The model under review builds one solid part; all positions refer to its coordinate system, in mm. Coordinates: 2 decimals unless noted, no trailing zeros. Order: outer loops, then holes, each group sorted by start corner. A loop starts at its lowest first (then second) coordinate and runs counter-clockwise, first axis right, second up. Notation, with made-up numbers: M -10.5,51.25 L 38.5,51.25 A26 cw 38.5,66.25 Z; hole C 78.5,47 d6. An arc over 180 degrees is marked long. Answer in a Markdown table with one row per item.
from build123d import *

# Parameters (mm, degrees)
BOSS_EXTRUDE1_DEPTH   = 7
SKETCH4_W             = 63
SKETCH4_H             = 38
CUT_EXTRUDE1_DEPTH    = 323.811382974
FILLET1_R             = 2
CUT_EXTRUDE2_DEPTH    = 323.811382974
FILLET2_R             = 2
M5_TAPPED_HOLE1_D     = 4.2
M5_TAPPED_HOLE1_DEPTH = 14
M5_TAPPED_HOLE1_TIP   = 1.2618073
M4_TAPPED_HOLE1_D     = 3.3
M4_TAPPED_HOLE1_DEPTH = 11.5
M4_TAPPED_HOLE1_TIP   = 0.991420021
FILLET3_R             = 3


with BuildPart() as part:
    # Sketch3 → Boss-Extrude1 (new, symmetric)
    with BuildSketch(Plane(origin=(50, 414.547428979, -101), x_dir=(0, 0, -1), z_dir=(-1, 0, 0))):
        Polygon((-101, 210.80448069), (-101, 290.80448069), (-262, 290.80448069), (-351, 227.80448069), (-351, 210.80448069), align=None)
    extrude(amount=BOSS_EXTRUDE1_DEPTH, both=True)

    # Sketch4 → Cut-Extrude1 (cut, through all)
    with BuildSketch(Plane(origin=(57, 0, 0), x_dir=(0, 0, -1), z_dir=(1, 0, 0))):
        with Locations((-46.5, 163.74294829)):
            Rectangle(SKETCH4_W, SKETCH4_H)
    extrude(amount=-CUT_EXTRUDE1_DEPTH, mode=Mode.SUBTRACT)

    # Fillet1
    fillet1_edges = [part.edges().sort_by_distance(p)[0] for p in [
        (50, 182.74294829, 15),
        (50, 144.74294829, 15),
        (50, 144.74294829, 78),
        (50, 182.74294829, 78),
    ]]
    fillet(fillet1_edges, radius=FILLET1_R)

    # Sketch5 → Cut-Extrude2 (cut, through all)
    with BuildSketch(Plane(origin=(57, 0, 0), x_dir=(0, 0, -1), z_dir=(1, 0, 0))):
        Polygon((-98, 144.74294829), (-157.507936508, 144.74294829), (-190, 167.74294829), (-190, 182.74294829), (-98, 182.74294829), align=None)
    extrude(amount=-CUT_EXTRUDE2_DEPTH, mode=Mode.SUBTRACT)

    # Fillet2
    fillet2_edges = [part.edges().sort_by_distance(p)[0] for p in [
        (50, 182.74294829, 98),
        (50, 144.74294829, 98),
        (50, 144.74294829, 157.507936508),
        (50, 167.74294829, 190),
        (50, 182.74294829, 190),
    ]]
    fillet(fillet2_edges, radius=FILLET2_R)

    # M5 Tapped Hole1
    with Locations(Plane(origin=(0, 0, 0), x_dir=(-1, 0, 0), z_dir=(0, 0, -1))):
        with Locations((-50.5, 188.74294829), (-50, 138.745448352)):
            Hole(M5_TAPPED_HOLE1_D / 2, depth=M5_TAPPED_HOLE1_DEPTH)
            with Locations((0, 0, -(M5_TAPPED_HOLE1_DEPTH + M5_TAPPED_HOLE1_TIP / 2))):  # 118° drill point
                Cone(0, M5_TAPPED_HOLE1_D / 2, M5_TAPPED_HOLE1_TIP, mode=Mode.SUBTRACT)

    # M4 Tapped Hole1
    with Locations(Plane(origin=(0, 203.74294829, 0), x_dir=(1, 0, 0), z_dir=(0, 1, 0))):
        with Locations((50, -114), (50, -174), (50, -234)):
            Hole(M4_TAPPED_HOLE1_D / 2, depth=M4_TAPPED_HOLE1_DEPTH)
            with Locations((0, 0, -(M4_TAPPED_HOLE1_DEPTH + M4_TAPPED_HOLE1_TIP / 2))):  # 118° drill point
                Cone(0, M4_TAPPED_HOLE1_D / 2, M4_TAPPED_HOLE1_TIP, mode=Mode.SUBTRACT)

    # Fillet3
    fillet3_edges = [part.edges().sort_by_distance(p)[0] for p in [
        (50, 186.74294829, 250),
        (50, 123.74294829, 161),
    ]]
    fillet(fillet3_edges, radius=FILLET3_R)


solid = part.part
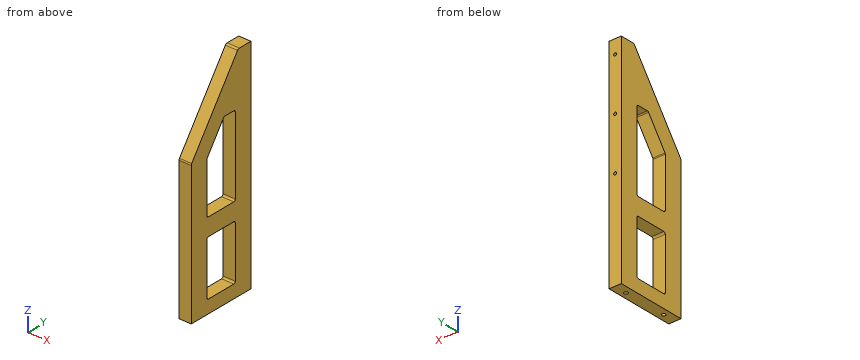
(1) Insertion check: P1, Ø7, axis at x = 53, y = 156, coming from the +Z side; P2, Ø4, axis at x = 50, z = 174, coming from the -Y side; P3, Ø4.5, axis at x = 50, z = 234, coming from the -Y side. Each pin has a flat end and moves straight along its axis. Give the tip position at first contact, or say it passes through.
Report:
| item | result |
|---|---|
| P1 | z = 211.51 |
| P2 | y = 131.53 |
| P3 | y = 173.82 |
(2) Take a section at A-A (z = 150). Write out the cut boundary in (x, y).
Report:
| item | result |
|---|---|
| outline | M 43,123.74 L 57,123.74 L 57,144.74 L 43,144.74 Z; M 43,182.74 L 57,182.74 L 57,203.74 L 43,203.74 Z |
(3) To check wall thickness, follow line 1 (Z direction, x = 50, y = 196.75); line 2 (Y direction, x = 50, z = 55); line 3 (Z direction, x = 54.5, y = 182). State the ranges of each line that lie inside material, in increasing order. Write a range as [from, to].
Report:
| item | result |
|---|---|
| line 1 | [0, 112.35], [115.65, 172.35], [175.65, 232.35], [235.65, 250] |
| line 2 | [123.74, 144.74], [182.74, 203.74] |
| line 3 | [0, 15.44], [77.56, 98.44], [189.56, 243.3] |
(4) Take a section at B-B (y = 177.5). Write out the cut boundary in (x, z).
Report:
| item | result |
|---|---|
| outline | M 43,0 L 57,0 L 57,15 L 43,15 Z; M 43,78 L 57,78 L 57,98 L 43,98 Z; M 43,190 L 57,190 L 57,236.94 L 43,236.94 Z |
